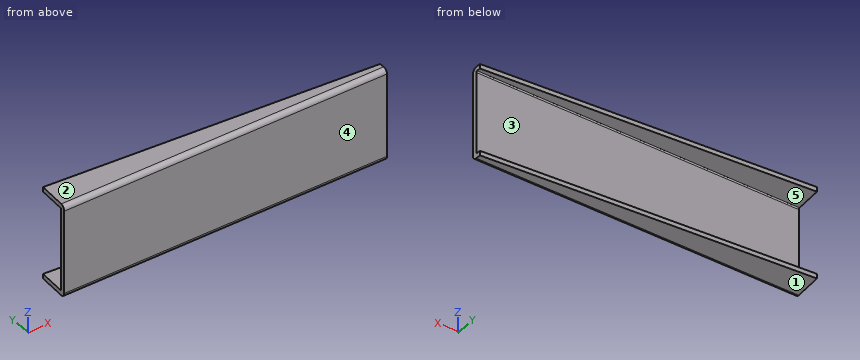
```python
from build123d import *

# Parameters (mm, degrees)
SKETCH_1_W          = 850
SKETCH_1_H          = 85
EXTRUDE_1_DEPTH     = 240
CUT_EXTRUDE_1_DEPTH = 240
SHELL_1_T           = -12
EXTRUDE_2_DEPTH     = 240
SKETCH_5_W          = 850
SKETCH_5_H          = 216
CUT_EXTRUDE_3_DEPTH = 94
FILLET_1_R          = 12
FILLET_2_R          = 3
CUT_EXTRUDE_4_DEPTH = 240


with BuildPart() as part:
    # 草图1 → 凸台-拉伸1 (new body)
    with BuildSketch(Plane.XY):
        Rectangle(SKETCH_1_W, SKETCH_1_H)
    extrude(amount=EXTRUDE_1_DEPTH)

    # 草图2 → 切除-拉伸1 (cut)
    with BuildSketch(Plane.XY.offset(240)):
        Polygon((-425, 42.5), (425, -17.5), (425, 42.5), align=None)
    extrude(amount=-CUT_EXTRUDE_1_DEPTH, mode=Mode.SUBTRACT)

    # 抽壳1
    shell_1_openings = [part.faces().sort_by_distance(p)[0] for p in [
        (425, -30, 120),
        (-425, 0, 120),
    ]]
    offset(amount=SHELL_1_T, openings=shell_1_openings, kind=Kind.INTERSECTION)

    # 草图6 → 凸台-拉伸2 (add)
    with BuildSketch(Plane(origin=(0, 0, 0), x_dir=(-1, 0, 0), z_dir=(0, 0, -1))):
        Polygon((425, 42.5), (431, -42.5), (425, -42.5), align=None)
    extrude(amount=-EXTRUDE_2_DEPTH)

    # 草图5 → 切除-拉伸3 (cut)
    with BuildSketch(Plane(origin=(0, -30.5, 0), x_dir=(1, 0, 0), z_dir=(0, 1, 0))):
        with Locations((0, -120)):
            Rectangle(SKETCH_5_W, SKETCH_5_H)
    extrude(amount=CUT_EXTRUDE_3_DEPTH, mode=Mode.SUBTRACT)

    # 圆角1
    fillet_1_edges = [part.edges().sort_by_distance(p)[0] for p in [
        (-3, -42.5, 0),
        (-3, -42.5, 240),
    ]]
    fillet(fillet_1_edges, radius=FILLET_1_R)

    # 圆角2
    fillet_2_edges = [part.edges().sort_by_distance(p)[0] for p in [
        (0, -30.5, 12),
        (0, -30.5, 228),
    ]]
    fillet(fillet_2_edges, radius=FILLET_2_R)

    # 草图7 → 切除-拉伸4 (cut)
    with BuildSketch(Plane(origin=(-425, 0, 0), x_dir=(0, 0, -1), z_dir=(1, 0, 0))):
        with BuildLine():
            Line((-225, -30.5), (-15, -30.5))
            ThreePointArc((-15, -30.5), (-12.878679656, -29.621320344), (-12, -27.5))
            Line((-12, -27.5), (-12, 42.5))
            Line((-12, 42.5), (-228, 42.5))
            Line((-228, 42.5), (-228, -27.5))
            ThreePointArc((-228, -27.5), (-227.121320344, -29.621320344), (-225, -30.5))
        make_face()
    extrude(amount=-CUT_EXTRUDE_4_DEPTH, mode=Mode.SUBTRACT)


solid = part.part
```
Part model, mm, in its own coordinate system. Face numbers are marked on the shaded views. A direction names the side the tool comes from. Round coordinates to 2 decimals unless told otherwise and drop trailing zeros. Write each loop counter-clockwise with the first axis right and the second up, starting at its lowest first coordinate (ties: lowest second). Pieces come first, ordered by that corner, then holes. Notation, with made-up numbers: (3.25, -27) -> (52.25, -27) arc R24 cw to (52.25, -7) -> close; hole circle Ø7 at (49, -23). An arc over 180 degrees is marked (long way). Return JSON: item names as keys, results as strings. Group by question number.
Q1. Saw through at B-B on y = 21.5. Write the cut outline in (x, z).
Q2. Pin check, flat tip, straight feed: pin 1 (12 mm diameter, centred on x = -179, z = 67, fed in from +Y). Stop position of the tip, or through.
Q3. Saw through at D-D on x = 155.5. Write the cut outline in (y, z).
Q4. Probe L1, parallel to Z at x = 46, y = -6.5; L2, parallel to Y at x = -298, z = 221.5; L3, parallel to Z at x = 375.5, y = -34.5. List the from-to ranges inside material, lowest first. Write a range as [from, to].
Q5. Saw through at A-A on x = -85. Write the cut outline in (y, z), plus the area to 3 significant figures.
Q6. Saw through at C-C on z = 113. Write the cut outline in (x, y).
Q7. Which spindle directions (+Z, -Z, +X, -X, +Y, -Y) get a long thin tool onto all of the face, cutting with end or side? Do the marked faces 4 and 5. Say none if no direction does.
Q8. Mould opens along Z. For the marked faces 1, 2 and 3 say: pulls with the +Z half, pulls with the -Z half, needs draft (parallel to the pull), parting line crosses it, or undercut.
Answer:
{
 "1": {"outline": "(-426.48, 0) -> (-127.5, 0) -> (-127.5, 12) -> (-426.48, 12) -> close; (-426.48, 228) -> (-127.5, 228) -> (-127.5, 240) -> (-426.48, 240) -> close"},
 "2": {"pin 1": "y = -30.5"},
 "3": {"outline": "(-42.5, 12) arc R12 ccw to (-30.5, 0) -> (1.52, 0) -> (1.52, 12) -> (-27.5, 12) arc R3 cw to (-30.5, 15) -> (-30.5, 225) arc R3 cw to (-27.5, 228) -> (1.52, 228) -> (1.52, 240) -> (-30.5, 240) arc R12 ccw to (-42.5, 228) -> close"},
 "4": {"L1": "[0, 12], [228, 240]", "L2": "[-42.5, -30.5]", "L3": "[0.69, 239.31]"},
 "5": {"outline": "(-42.5, 12) arc R12 ccw to (-30.5, 0) -> (18.5, 0) -> (18.5, 12) -> (-27.5, 12) arc R3 cw to (-30.5, 15) -> (-30.5, 225) arc R3 cw to (-27.5, 228) -> (18.5, 228) -> (18.5, 240) -> (-30.5, 240) arc R12 ccw to (-42.5, 228) -> close", "area": "4,000 mm2"},
 "6": {"outline": "(-431, -42.5) -> (425, -42.5) -> (425, -30.5) -> (-430.15, -30.5) -> close"},
 "7": {"face 4": "+Z, -Z, +X, -X, -Y", "face 5": "+X, -X, +Y"},
 "8": {"face 1": "pulls with the -Z half", "face 2": "pulls with the +Z half", "face 3": "undercut"}
}
